CAD build for the part. Positions are in the model's coordinates, mm. A direction names the side the tool comes from. Round coordinates to 2 decimals unless told otherwise and drop trailing zeros. Order: outer loops, then holes, each group sorted by start corner. A loop starts at its lowest first (then second) coordinate and runs counter-clockwise, first axis right, second up.
```python
from build123d import *

# Parameters (mm, degrees)
ROUND_FLANGE_SKETCH_R          = 49
ROUND_FLANGE_98_DEPTH          = 15
ROUND_FLANGE_HOLES_SKETCH_R    = 5
ROUND_FLANGE_HOLES_6X_10_DEPTH = 15
SLEEVE_SKETCH_R                = 25
SLEEVE_50_DEPTH                = 60
OVAL_FLANGE_DEPTH              = 15
OVAL_FLANGE_HOLES_SKETCH_R     = 6
OVAL_FLANGE_HOLES_2X_12_DEPTH  = 15
COUNTERBORE_SKETCH_R           = 17.5
COUNTERBORE_35_DEPTH           = 30
BORE_SKETCH_R                  = 14
BORE_28_DEPTH                  = 45


with BuildPart() as part:
    # Round Flange Sketch → Round Flange Ø98 (new body)
    with BuildSketch(Plane.XY):
        Circle(ROUND_FLANGE_SKETCH_R)
    extrude(amount=ROUND_FLANGE_98_DEPTH)

    # Round Flange Holes Sketch → Round Flange Holes 6xØ10 (cut)
    with BuildSketch(Plane.XY.offset(15)):
        with Locations((0, 35)):
            Circle(ROUND_FLANGE_HOLES_SKETCH_R)
        with Locations((30.310889132, 17.5)):
            Circle(ROUND_FLANGE_HOLES_SKETCH_R)
        with Locations((30.310889132, -17.5)):
            Circle(ROUND_FLANGE_HOLES_SKETCH_R)
        with Locations((0, -35)):
            Circle(ROUND_FLANGE_HOLES_SKETCH_R)
        with Locations((-30.310889132, -17.5)):
            Circle(ROUND_FLANGE_HOLES_SKETCH_R)
        with Locations((-30.310889132, 17.5)):
            Circle(ROUND_FLANGE_HOLES_SKETCH_R)
    extrude(amount=-ROUND_FLANGE_HOLES_6X_10_DEPTH, mode=Mode.SUBTRACT)

    # Sleeve Sketch → Sleeve Ø50 (add)
    with BuildSketch(Plane.XY.offset(15)):
        Circle(SLEEVE_SKETCH_R)
    extrude(amount=SLEEVE_50_DEPTH)

    # Oval Flange Sketch → Oval Flange (add)
    with BuildSketch(Plane.XY.offset(75)):
        with BuildLine():
            Line((-14.812486777, -54.633777367), (-28.714375061, -8.688191115))
            ThreePointArc((-28.714375061, -8.688191115), (-29.999971167, 0.041592963), (-28.690173521, 8.7677787))
            Line((-28.690173521, 8.7677787), (-14.786489776, 54.263806016))
            ThreePointArc((-14.786489776, 54.263806016), (-0.706868372, 65.68836713), (14.083896835, 55.200774455))
            Line((14.083896835, 55.200774455), (28.617323634, 9.002710037))
            ThreePointArc((28.617323634, 9.002710037), (29.999548575, 0.16457607), (28.714375061, -8.688191115))
            Line((28.714375061, -8.688191115), (14.812486777, -54.633777367))
            ThreePointArc((14.812486777, -54.633777367), (0, -65.627604906), (-14.812486777, -54.633777367))
        make_face()
    extrude(amount=OVAL_FLANGE_DEPTH)

    # Oval Flange Holes Sketch → Oval Flange Holes 2xØ12 (cut)
    with BuildSketch(Plane.XY.offset(90)):
        with Locations((-0.220456426, 50.700774863)):
            Circle(OVAL_FLANGE_HOLES_SKETCH_R)
        with Locations((0, -50.151920606)):
            Circle(OVAL_FLANGE_HOLES_SKETCH_R)
    extrude(amount=-OVAL_FLANGE_HOLES_2X_12_DEPTH, mode=Mode.SUBTRACT)

    # Counterbore Sketch → Counterbore Ø35 (cut)
    with BuildSketch(Plane.XY.offset(90)):
        Circle(COUNTERBORE_SKETCH_R)
    extrude(amount=-COUNTERBORE_35_DEPTH, mode=Mode.SUBTRACT)

    # Bore Sketch → Bore Ø28 (cut)
    with BuildSketch(Plane.XY.offset(60)):
        Circle(BORE_SKETCH_R)
    extrude(amount=-BORE_28_DEPTH, mode=Mode.SUBTRACT)


solid = part.part
```
1. Cut at B-B, the plane y = -35. Write the cut outline in (x, z).
2. Mould opens along X. For faces 1 (the face through (-13, -14, 90)), 2 (the face through (0, 0, 15)), 3 (the face through (21.86, -31.34, 82.4)) say: released by +X, released by -X, zero draft, split by the parting line, or undercut.
3. Cut at C-C, the plane z = 73. Write the cut outline in (x, y).
4. Pin check, flat tips, straight feed: P1, Ø1, axis at y = -32, z = 12, coming from the -X side; P2, Ø7, axis at x = 0, y = -50.15, coming from the +Z side; P3, Ø6, axis at x = -6, z = 65, coming from the +Y side; P4, Ø6, axis at x = -30.31, y = 17.5, coming from the +Z side (3 decimals). Stop position of each tip, or through.
5. Drill centre lines: line 1 (Z direction, x = -25, y = 7); line 2 (Y direction, x = 0, z = 27); line 3 (X direction, y = -37, z = 6). Where is each one in solid material? Low to high.
6. Cut at D-D, the plane x = 42.5. Write the cut outline in (y, z), and give its area (3 significant figures).
7. Tool access for faces 4 (the face through (-1.521, 44.843, 82.605)), 5 (the face through (-1.08, -39.88, 7.6)), 6 (the face through (30, 0, 82)): list every direction of +Z, -Z, +X, -X, +Y, -Y with a clear straight run to the whole face (end or side of a thin tool).
8. Cut at A-A, the plane y = 0. Write the cut outline in (x, z), and give its area (3 significant figures).
Outcome:
1. outline: (-34.29, 0) - (-5, 0) - (-5, 15) - (-34.29, 15) - close; (-20.75, 75) - (20.75, 75) - (20.75, 90) - (-20.75, 90) - close; (5, 0) - (34.29, 0) - (34.29, 15) - (5, 15) - close
2. face 1: zero draft
2. face 2: undercut
2. face 3: released by +X
3. outline: circle Ø50 at (0, 0); hole circle Ø35 at (0, 0)
4. P1: stops at x = -37.53
4. P2: stops at z = 15
4. P3: stops at y = 24.82
4. P4: passes through
5. line 1: z = 0 to 15, 75 to 90
5. line 2: y = -25 to -14, 14 to 25
5. line 3: x = -32.12 to -4.58, 4.58 to 32.12
6. outline: (-24.39, 0) - (24.39, 0) - (24.39, 15) - (-24.39, 15) - close
6. area: 732 mm2
7. face 4: +Z
7. face 5: -Z
7. face 6: +Z, +X
8. outline: (-49, 0) - (49, 0) - (49, 15) - (25, 15) - (25, 75) - (30, 75) - (30, 90) - (17.5, 90) - (17.5, 60) - (14, 60) - (14, 15) - (-14, 15) - (-14, 60) - (-17.5, 60) - (-17.5, 90) - (-30, 90) - (-30, 75) - (-25, 75) - (-25, 15) - (-49, 15) - close
8. area: 3,060 mm2
